Can you work these out from the model? Positions are in its coordinate system, mm. A direction names the side the tool comes from. Give positions to 0.01 mm unless a question says otherwise; leave off trailing zeros. Write each loop counter-clockwise with the first axis right and the second up, starting at its lowest first coordinate (ties: lowest second). Pieces come first, ordered by that corner, then holes. Notation, with made-up numbers: M -19.75,83 L 7.25,83 A16 cw 7.25,90 Z; hole C 48.25,50.25 d9. An arc over 180 degrees is marked long. Use CSV: the item, a comma, the result in double quotes. Start each with the question number.
from build123d import *

# Parameters (mm, degrees)
SKETCH_1_R          = 1.5
EXTRUDE_1_DEPTH     = 13
CUT_EXTRUDE_3_DEPTH = 7
CUT_EXTRUDE_4_DEPTH = 7
SKETCH_3_R          = 1.75
CUT_EXTRUDE_2_DEPTH = 22.100947846


with BuildPart() as part:
    # 草图1 → 凸台-拉伸1 (new, symmetric)
    with BuildSketch(Plane.XY):
        with BuildLine():
            Line((-2.598076211, -1.5), (-16, -1.5))
            Line((-16, -1.5), (-16, -3))
            Line((-16, -3), (0, -3))
            ThreePointArc((0, -3), (1.5, 2.598076211), (-2.598076211, -1.5))
        make_face()
        with Locations(Location((0, 0, 0), (0, 0, 180))):
            Circle(SKETCH_1_R, mode=Mode.SUBTRACT)
    extrude(amount=EXTRUDE_1_DEPTH, both=True)

    # 草图2 → 切除-拉伸3 (cut)
    with BuildSketch(Plane.XY.offset(13)):
        with BuildLine():
            Line((-3.5, 0), (-3.5, -3))
            Line((-3.5, -3), (-1.802775638, -3))
            ThreePointArc((-1.802775638, -3), (3.046285831, 1.723410176), (-3.5, 0))
        make_face()
    extrude(amount=-CUT_EXTRUDE_3_DEPTH, mode=Mode.SUBTRACT)

    # 草图4 → 切除-拉伸4 (cut)
    with BuildSketch(Plane(origin=(0, 0, -13), x_dir=(-1, 0, 0), z_dir=(0, 0, -1))):
        with BuildLine():
            Line((3.5, -3), (3.5, 0))
            ThreePointArc((3.5, 0), (-3.046285831, 1.723410176), (1.802775638, -3))
            Line((1.802775638, -3), (3.5, -3))
        make_face()
    extrude(amount=-CUT_EXTRUDE_4_DEPTH, mode=Mode.SUBTRACT)

    # 草图3 → 切除-拉伸2 (cut, through all)
    with BuildSketch(Plane(origin=(0, -1.5, 0), x_dir=(1, 0, 0), z_dir=(0, 1, 0))):
        with Locations(Location((-11, 6.5, 0), (0, 0, 180))):
            Circle(SKETCH_3_R)
        with Locations((-11, -6.5)):
            Circle(SKETCH_3_R)
    extrude(amount=-CUT_EXTRUDE_2_DEPTH, mode=Mode.SUBTRACT)


solid = part.part
(1) Which directions (+Z, -Z, +X, -X, +Y, -Y) give clear straight access to the entire face, cutting with the end or side of a thin tool? Please do faces 1 (the face through (-3.5, -2, -10)), 2 (the face through (-2, 0, 6)), 3 (the face through (-11.81, -2.24, -8.05)).
(2) Thinking about a two-plate mould opening in X: for faces 4 (the face through (-3.5, -2, 10)), 5 (the face through (-2, 0, -6)), 6 (the face through (-1.43, -0.45, -0.08)), which applies, released by +X, released by -X, zero draft, split by the parting line, or undercut?
(3) Please list where these lines run through material, in increasing order: L1, parallel to Z at x = -11, y = -2.45; L2, parallel to X at y = -1.95, z = 6.5; L3, parallel to Y at x = -5, z = -4.75. Write a range as [from, to].
(4) I want a section at C-C (z = -6.5). Write out the boundary of the cut face in (x, y).
(5) I want a section at B-B (x = -11). Write out the boundary of the cut face in (y, z).
(6) Will these pins go through, and if not, where does the flat tip stop? pin 1 Ø10.5 at (x, z) = (-12.5, 3.5) entering from +Y; pin 2 Ø8 at (x, z) = (-5.5, 7) entering from +Y; pin 3 Ø3.5 at (x, y) = (0, 0) entering from +Z.
(7) I want a section at A-A (y = 0). Write out the boundary of the cut face in (x, z).
(8) I want a section at D-D (y = -2). Write out the boundary of the cut face in (x, z).
Geometry results:
1,face 1,"-Z, +X, +Y, -Y"
1,face 2,"+Z, +X, +Y, -Y"
1,face 3,"+Y, -Y"
2,face 4,"released by +X"
2,face 5,"zero draft"
2,face 6,"undercut"
3,L1,"z = [-13, -8.25], [-4.75, 4.75], [8.25, 13]"
3,L2,"x = [-16, -12.75], [-9.25, -3.5]"
3,L3,"y = [-3, -1.5]"
4,outline,"M -16,-3 L -12.75,-3 L -12.75,-1.5 L -16,-1.5 Z; M -9.25,-3 L -3.5,-3 L -3.5,-1.5 L -9.25,-1.5 Z"
5,outline,"M -3,-13 L -1.5,-13 L -1.5,-8.25 L -3,-8.25 Z; M -3,-4.75 L -1.5,-4.75 L -1.5,4.75 L -3,4.75 Z; M -3,8.25 L -1.5,8.25 L -1.5,13 L -3,13 Z"
6,pin 1,"stops at y = -1.5"
6,pin 2,"stops at y = 2.52"
6,pin 3,"stops at z = 6"
7,outline,"M -3,-6 L -1.5,-6 L -1.5,6 L -3,6 Z; M 1.5,-6 L 3,-6 L 3,6 L 1.5,6 Z"
8,outline,"M -16,-13 L -3.5,-13 L -3.5,-6 L 2.24,-6 L 2.24,6 L -3.5,6 L -3.5,13 L -16,13 Z; hole C -11,-6.5 d3.5; hole C -11,6.5 d3.5"
